```python
from build123d import *

# Parameters (mm, degrees)
SKETCH_1_W                   = 71
SKETCH_1_H                   = 10
EXTRUDE_1_DEPTH              = 43.6
HOLE_WIZARD_M4_1_D           = 4.5
HOLE_WIZARD_M4_1_CBORE_D     = 8
HOLE_WIZARD_M4_1_CBORE_DEPTH = 4.6
HOLE_WIZARD_M4_1_2_D         = 3.3
HOLE_WIZARD_M4_1_2_DEPTH     = 10.1
HOLE_WIZARD_M4_1_2_TIP       = 0.991420021


with BuildPart() as part:
    # 草图1 → 凸台-拉伸1 (new body)
    with BuildSketch(Plane(origin=(0, 0, 0), x_dir=(1, 0, 0), z_dir=(0, 1, 0))):
        with Locations((35.5, 5)):
            Rectangle(SKETCH_1_W, SKETCH_1_H)
    extrude(amount=EXTRUDE_1_DEPTH)

    # Hole Wizard M4 _1 (through all)
    with Locations(Plane(origin=(0, 0, -10), x_dir=(-1, 0, 0), z_dir=(0, 0, -1))):
        with Locations((-66, 36.8), (-66, 21.783451384), (-66, 6.8)):
            CounterBoreHole(HOLE_WIZARD_M4_1_D / 2, HOLE_WIZARD_M4_1_CBORE_D / 2, HOLE_WIZARD_M4_1_CBORE_DEPTH)

    # Hole Wizard M4 _1 2
    with Locations(Plane.ZY):
        with Locations((-5, 37.8), (-5, 21.8), (-5, 5.8)):
            Hole(HOLE_WIZARD_M4_1_2_D / 2, depth=HOLE_WIZARD_M4_1_2_DEPTH)
            with Locations((0, 0, -(HOLE_WIZARD_M4_1_2_DEPTH + HOLE_WIZARD_M4_1_2_TIP / 2))):  # 118° drill point
                Cone(0, HOLE_WIZARD_M4_1_2_D / 2, HOLE_WIZARD_M4_1_2_TIP, mode=Mode.SUBTRACT)


solid = part.part
```
Geometry check sheet. Reference: the model listing, model coordinates, mm. A direction names the side the tool comes from. Round coordinates to 2 decimals unless told otherwise and drop trailing zeros. Order: outer loops, then holes, each group sorted by start corner. A loop starts at its lowest first (then second) coordinate and runs counter-clockwise, first axis right, second up. Notation, with made-up numbers: M 18,41 L 38,41 A11 cw 38,52 Z; hole C -9,66.5 d9. An arc over 180 degrees is marked long. Answer as CSV lines item,"result".
1) Sectioned sample at A-A on x = 66. Record the cut outline in (y, z), and give its area (3 significant figures).
Entries:
outline,"M 0,-10 L 2.8,-10 L 2.8,-5.4 L 4.55,-5.4 L 4.55,0 L 0,0 Z; M 9.05,-5.4 L 10.8,-5.4 L 10.8,-10 L 17.78,-10 L 17.78,-5.4 L 19.53,-5.4 L 19.53,0 L 9.05,0 Z; M 24.03,-5.4 L 25.78,-5.4 L 25.78,-10 L 32.8,-10 L 32.8,-5.4 L 34.55,-5.4 L 34.55,0 L 24.03,0 Z; M 39.05,-5.4 L 40.8,-5.4 L 40.8,-10 L 43.6,-10 L 43.6,0 L 39.05,0 Z"
area,"253 mm2"
2) Thickness scan on probe 1 along Y at (x, z) = (66, -1.9); probe 2 along Y at (x, z) = (6.75, -5); probe 3 along X at (y, z) = (22, -2.5). Record the ranges inside material, lowest first. Write a range as [from, to].
Entries:
probe 1,"[0, 4.55], [9.05, 19.53], [24.03, 34.55], [39.05, 43.6]"
probe 2,"[0, 4.15], [7.45, 20.15], [23.45, 36.15], [39.45, 43.6]"
probe 3,"[0, 63.76], [68.24, 71]"
3) Gauge pin test, flat ends, axial feed: pin 1 Ø4 at (x, y) = (66, 36.8) entering from +Z; pin 2 Ø4 at (x, y) = (67, 38) entering from -Z; pin 3 Ø4 at (x, y) = (43.5, 27) entering from +Z; pin 4 Ø2.5 at (y, z) = (37.8, -5) entering from -X. Record the tip position at first contact, or that the pin passes through.
Entries:
pin 1,"through"
pin 2,"z = -5.4"
pin 3,"z = 0"
pin 4,"x = 10.34"
4) Sectioned sample at B-B on z = -1.75. Record the cut outline in (x, y).
Entries:
outline,"M 0,0 L 71,0 L 71,43.6 L 0,43.6 Z; hole C 66,6.8 d4.5; hole C 66,21.78 d4.5; hole C 66,36.8 d4.5"
5) Tool access check on faces 1 (the face through (64, 35, -5.4)), 2 (the face through (5.121, 38.915, -3.784)), 3 (the face through (63.752, 6.899, -2.662)). Record the directions out of +Z, -Z, +X, -X, +Y, -Y that give a thin tool (end or side, any length) a straight path to the whole face; none if there is none.
Entries:
face 1,"-Z"
face 2,"-X"
face 3,"+Z, -Z"
6) Mould release check, pull along X, two halves, no side actions. Record for faces 4 (the face through (62.185, 38.001, -7.732)), 5 (the face through (71, 21, -5)), 6 (the face through (10.92, 5.63, -5.23)), 7 (the face through (35, 43.6, -5)): +X half, -X half, draft (parallel to the pull), parting line (faces both ways), or undercut.
Entries:
face 4,"undercut"
face 5,"+X half"
face 6,"-X half"
face 7,"draft"
